For this review, take the finished solid that the model builds, in its own axes (mm). Coordinates: 2 decimals unless noted, no trailing zeros. Order: outer loops, then holes, each group sorted by start corner. A loop starts at its lowest first (then second) coordinate and runs counter-clockwise, first axis right, second up. Notation, with made-up numbers: (87.25, 5) -> (101.25, 5) arc R11 cw to (101.25, 10) -> close; hole circle Ø10 at (73.25, 52.25). An arc over 180 degrees is marked (long way). Write item = value, one per line. Start each with the question number.
1) Consider section A-A on x = 33. Give the boundary of the cut face in (y, z), and give its area (3 significant figures).
2) Draft analysis for pull direction Z (two halves, no side actions). For faces 1 (the face through (18, 28, 0)), 2 (the face through (18, 28, 3)), 3 (the face through (33, 53, 1)), state which applies: +Z half, -Z half, draft (parallel to the pull), parting line (faces both ways), or undercut.
3) Wall thickness on probe 1 along Y at (x, z) = (32.5, 2.8); probe 2 along X at (y, z) = (52, 1.8): over which ranges is each line inside the solid? List them lowest first. Write a range as [from, to].
from build123d import *

# Parameters (mm, degrees)
SKETCH_1_W      = 36
SKETCH_1_H      = 55
EXTRUDE_1_DEPTH = 3
CHAMFER_1_SIZE  = 5


with BuildPart() as part:
    # 草图1 → 凸台-拉伸1 (new body)
    with BuildSketch(Plane.XY):
        with Locations((18, 27.5)):
            Rectangle(SKETCH_1_W, SKETCH_1_H)
    extrude(amount=EXTRUDE_1_DEPTH)

    # 倒角1
    chamfer_1_edges = [part.edges().sort_by_distance(p)[0] for p in [
        (36, 55, 1.5),
        (36, 0, 1.5),
    ]]
    chamfer(chamfer_1_edges, length=CHAMFER_1_SIZE)


solid = part.part
Answer sheet:
q1.outline = (2, 0) -> (53, 0) -> (53, 3) -> (2, 3) -> close
q1.area = 153 mm2
q2.face_1 = -Z half
q2.face_2 = +Z half
q2.face_3 = draft
q3.probe_1 = [1.5, 53.5]
q3.probe_2 = [0, 34]
